The figure shows three views and two pictorial views of one solid part (mm, origin at its lowest corner). Answer the questions. Give positions to 0.01 mm unless a question says otherwise; leave off trailing zeros. Loops run counter-clockwise (first coordinate to the right, second up) from the corner with the lowest first, then second, coordinate; pieces in that order, holes last. Notation, with made-up numbers: M 66,-0.75 L 117,-0.75 A18 cw 117,25.25 Z; hole C -7,23.25 d8. An arc over 180 degrees is marked long. One line per item, written item: value. Start each with the question number.
Q1. A cutting plane is placed at A-A, the plane x = 25. Determine the outline of the cut face in (y, z).
Q2. Flat-ended cylindrical pins translate along their axes: pin 1 (1 mm diameter, centred on x = 16, z = 7, fed in from -Y); pin 2 (6 mm diameter, centred on x = 25, y = 25, fed in from -Z). Find the tip coordinate at first contact, or state that the pin passes through.
Q3. A cutting plane is placed at C-C, the plane z = 3.25. Determine the outline of the cut face in (x, y).
Q4. Consider L1, parallel to Y at x = 25, z = 4; L2, parallel to X at y = 25.5, z = 2.25; L3, parallel to Y at x = 22.5, z = 1.5. Determine where each line is inside the solid, lowest interval first.
Q5. The mould has two halves that part along Y. Classify the marked faces 1, 2 and 3: +Y half, -Y half, draft (parallel to the pull), parting line (faces both ways), or undercut.
Q6. A cutting plane is placed at B-B, the plane y = 105. Determine the outline of the cut face in (x, z).
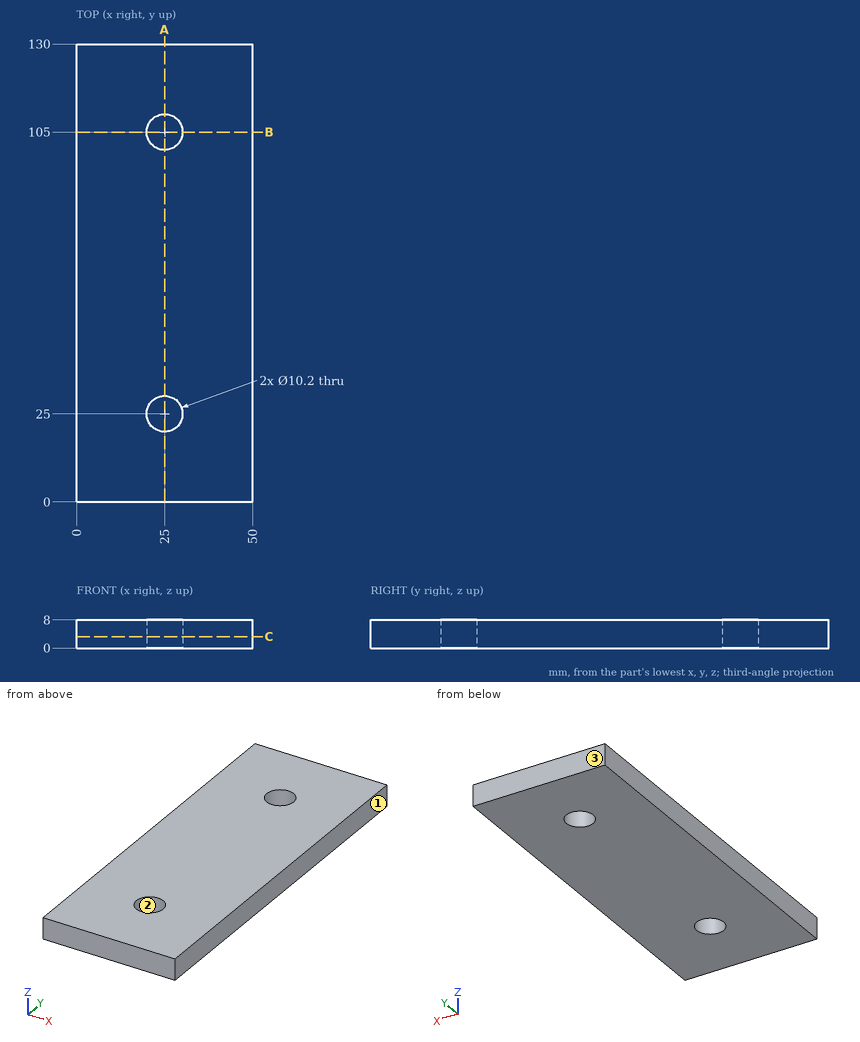
Answer block:
1. outline: M 0,0 L 19.9,0 L 19.9,8 L 0,8 Z; M 30.1,0 L 99.9,0 L 99.9,8 L 30.1,8 Z; M 110.1,0 L 130,0 L 130,8 L 110.1,8 Z
2. pin 1: y = 0
2. pin 2: through
3. outline: M 0,0 L 50,0 L 50,130 L 0,130 Z; hole C 25,25 d10.2; hole C 25,105 d10.2
4. L1: 0 to 19.9, 30.1 to 99.9, 110.1 to 130
4. L2: 0 to 19.92, 30.08 to 50
4. L3: 0 to 20.55, 29.45 to 100.55, 109.45 to 130
5. face 1: draft
5. face 2: undercut
5. face 3: +Y half
6. outline: M 0,0 L 19.9,0 L 19.9,8 L 0,8 Z; M 30.1,0 L 50,0 L 50,8 L 30.1,8 Z
